Geometry check sheet. Reference: the model listing, model coordinates, mm. Coordinates: 2 decimals unless noted, no trailing zeros. Loops run counter-clockwise (first coordinate to the right, second up) from the corner with the lowest first, then second, coordinate; pieces in that order, holes last.
from build123d import *

# Parameters (mm, degrees)
BOSS_EXTRUDE1_DEPTH = 0.2


with BuildPart() as part:
    # Sketch1 → Boss-Extrude1 (new body)
    with BuildSketch(Plane(origin=(0, 0, 0), x_dir=(1, 0, 0), z_dir=(0, 1, 0))):
        Polygon((14.2, 1.7), (18.405344965, 6.07), (19.5, 6.07), (19.5, 5.72), (18.5, 5.72), (14.095006994, 0), (0, 0), (0, 1.7), align=None)
    extrude(amount=BOSS_EXTRUDE1_DEPTH)


solid = part.part
(1) Scan lines: L1, parallel to Z at x = 2.5, y = 0.15; L2, parallel to X at y = 0.1, z = -4.5; L3, parallel to X at y = 0.1, z = -5. Record each from-to range of solid material in increasing order.
Findings:
L1: z = -1.7 to 0
L2: x = 16.89 to 17.56
L3: x = 17.38 to 17.95
(2) Sectioned sample at A-A on y = 0.05. Record the cut outline in (x, z) (3 decimals), and give its area (3 significant figures).
Findings:
outline: (0, -1.7) - (14.2, -1.7) - (18.405, -6.07) - (19.5, -6.07) - (19.5, -5.72) - (18.5, -5.72) - (14.095, 0) - (0, 0) - close
area: 28.8 mm2
(3) Gauge pin test, flat end, axial feed: pin 1 Ø1 at (x, z) = (9.5, -3) entering from -Y. Record the tip position at first contact, or that the pin passes through.
Findings:
pin 1: passes through
(4) Sectioned sample at C-C on z = -0.75. Record the cut outline in (x, y).
Findings:
outline: (0, 0) - (14.67, 0) - (14.67, 0.2) - (0, 0.2) - close
(5) Draft check along Y on faces 1 (the flat face through (9, 0.2, -1)), 2 (the flat face through (9, 0, -1)). Enter one of: +Y half, -Y half, draft (parallel to the pull), parting line (faces both ways), or undercut.
Findings:
face 1: +Y half
face 2: -Y half
(6) Sectioned sample at B-B on x = 1.75. Record the cut outline in (y, z), and give its area (3 significant figures).
Findings:
outline: (0, -1.7) - (0.2, -1.7) - (0.2, 0) - (0, 0) - close
area: 0.340 mm2
